from build123d import *

# Parameters (mm, degrees)
BOSS_EXTRUDE1_DEPTH = 10


with BuildPart() as part:
    # Sketch1 → Boss-Extrude1 (new body)
    with BuildSketch(Plane.XY):
        with BuildLine():
            Line((-16, 50), (-28, 50))
            Line((-28, 50), (-28, 15))
            Line((-28, 15), (-46, 15))
            Line((-46, 15), (-46, 0))
            Line((-46, 0), (46, 0))
            Line((46, 0), (46, 15))
            Line((46, 15), (28, 15))
            Line((28, 15), (28, 50))
            Line((28, 50), (16, 50))
            ThreePointArc((16, 50), (0, 34), (-16, 50))
        make_face()
    extrude(amount=BOSS_EXTRUDE1_DEPTH)


solid = part.part
Part model, mm, in its own coordinate system. A direction names the side the tool comes from. Coordinates: 2 decimals unless noted, no trailing zeros. Write each loop counter-clockwise with the first axis right and the second up, starting at its lowest first coordinate (ties: lowest second). Pieces come first, ordered by that corner, then holes. Notation, with made-up numbers: M -21,23 L -13,23 A21 cw -13,36 Z; hole C 59,26.25 d5. An arc over 180 degrees is marked long. Return JSON: item names as keys, results as strings.
1. Saw through at B-B, the plane y = 41.5. Write the cut outline in (x, z).
Determined:
{"outline": "M -28,0 L -13.56,0 L -13.56,10 L -28,10 Z; M 13.56,0 L 28,0 L 28,10 L 13.56,10 Z"}
2. Probe L1, parallel to X at y = 22, z = 1.25; L2, parallel to Y at x = 28.5, z = 2.75; L3, parallel to Y at x = -0.5, z = 0.5. List the from-to ranges inside material, lowest first.
Determined:
{"L1": "-28 to 28", "L2": "0 to 15", "L3": "0 to 34.01"}
3. Saw through at C-C, the plane x = 37. Write the cut outline in (y, z), then the cut area to 3 significant figures.
Determined:
{"outline": "M 0,0 L 15,0 L 15,10 L 0,10 Z", "area": "150 mm²"}
4. Saw through at A-A, the plane z = 3.25. Write the cut outline in (x, y).
Determined:
{"outline": "M -46,0 L 46,0 L 46,15 L 28,15 L 28,50 L 16,50 A16 cw -16,50 L -28,50 L -28,15 L -46,15 Z"}
5. Saw through at D-D, the plane y = 28. Write the cut outline in (x, z).
Determined:
{"outline": "M -28,0 L 28,0 L 28,10 L -28,10 Z"}
6. 3-axis set-ups, long thin cutter, end or side, ignore diameter. For faces 5 (the face through (37, 15, 5)), 6 (the face through (-37, 15, 5)), 7 (the face through (-22, 50, 5)): which of +Z, -Z, +X, -X, +Y, -Y reach the whole face in a straight line?
Determined:
{"face 5": "+Z, -Z, +X, +Y", "face 6": "+Z, -Z, -X, +Y", "face 7": "+Z, -Z, +X, -X, +Y"}
7. Flat gauge pins, fed straight in: pin 1 Ø3 at (y, z) = (39, 8.5) entering from +X; pin 2 Ø3 at (y, z) = (26, 7.5) entering from -X; pin 3 Ø3 at (x, z) = (-7.5, 5.5) entering from -Y; pin 4 Ø3 at (x, z) = (35.5, 6) entering from +Y. Where does each tip first touch, or does it go through?
Determined:
{"pin 1": "x = 28", "pin 2": "x = -28", "pin 3": "y = 0", "pin 4": "y = 15"}
8. Pull direction X, two halves, no side cores. Call faces 1 (the face through (0, 34, 5)), 2 (the face through (28, 32, 5)), 3 (the face through (-46, 8, 5)), 4 (the face through (22, 50, 5)): pulls with the +X half, pulls with the -X half, needs draft (parallel to the pull), parting line crosses it, or undercut.
Determined:
{"face 1": "undercut", "face 2": "pulls with the +X half", "face 3": "pulls with the -X half", "face 4": "needs draft"}
